from build123d import *

# Parameters (mm, degrees)
BASE_PLATE_184X82X17_DEPTH      = 17
BEARING_SADDLE_DEPTH            = 45
RAISED_PAD_DEPTH                = 82
STEP_PROFILE_DEPTH              = 82
SLOT_CUT_DEPTH                  = 82
BOLT_BOSSES_SKETCH_R            = 9
BOLT_BOSSES_2X_WITH_HOLES_DEPTH = 39
END_BLOCK_DEPTH                 = 26


with BuildPart() as part:
    # Base Plate Sketch → Base Plate 184x82x17 (new body)
    with BuildSketch(Plane(origin=(0, 0, 0), x_dir=(1, 0, 0), z_dir=(0, 1, 0))):
        with BuildLine():
            Line((-86, -41), (92, -41))
            Line((92, -41), (92, 41))
            Line((92, 41), (-86, 41))
            ThreePointArc((-86, 41), (-90.242640687, 39.242640687), (-92, 35))
            Line((-92, 35), (-92, -35))
            ThreePointArc((-92, -35), (-90.242640687, -39.242640687), (-86, -41))
        make_face()
    extrude(amount=BASE_PLATE_184X82X17_DEPTH)

    # Bearing Saddle Sketch → Bearing Saddle (add)
    with BuildSketch(Plane(origin=(0, 17, 0), x_dir=(1, 0, 0), z_dir=(0, 1, 0))):
        with BuildLine():
            Line((92, -41), (56, -41))
            ThreePointArc((56, -41), (51.757359313, -39.242640687), (50, -35))
            Line((50, -35), (50, 35))
            ThreePointArc((50, 35), (51.757359313, 39.242640687), (56, 41))
            Line((56, 41), (92, 41))
            Line((92, 41), (92, -41))
        make_face()
    extrude(amount=BEARING_SADDLE_DEPTH)

    # Raised Pad Sketch → Raised Pad (add)
    with BuildSketch(Plane.XY.offset(41)):
        with BuildLine():
            Line((-58, 17), (-58, 0))
            Line((-58, 0), (-38, 0))
            Line((-38, 0), (-38, 17))
            ThreePointArc((-38, 17), (-48, 27), (-58, 17))
        make_face()
    extrude(amount=-RAISED_PAD_DEPTH)

    # Step Profile Sketch → Step Profile (add)
    with BuildSketch(Plane.XY.offset(41)):
        with BuildLine():
            Line((-64, 17), (-58, 17))
            ThreePointArc((-58, 17), (-48, 27), (-38, 17))
            Line((-38, 17), (-32, 17))
            ThreePointArc((-32, 17), (-48, 33), (-64, 17))
        make_face()
    extrude(amount=-STEP_PROFILE_DEPTH)

    # Slot Cut Sketch → Slot Cut (cut)
    with BuildSketch(Plane.XY.offset(41)):
        with BuildLine():
            Line((-58, 17), (-58, 0))
            Line((-58, 0), (-38, 0))
            Line((-38, 0), (-38, 17))
            ThreePointArc((-38, 17), (-48, 27), (-58, 17))
        make_face()
    extrude(amount=-SLOT_CUT_DEPTH, mode=Mode.SUBTRACT)

    # Bolt Bosses Sketch → Bolt Bosses 2x with Holes (add)
    # profile 1 of 2: a face of its own
    with BuildSketch(Plane(origin=(0, 17, 0), x_dir=(1, 0, 0), z_dir=(0, 1, 0))):
        with BuildLine():
            Line((32, 41), (56, 41))
            Line((56, 41), (56, 5))
            Line((56, 5), (32, 5))
            ThreePointArc((32, 5), (14, 23), (32, 41))
        make_face()
        with Locations(Location((32, 23, 0), (0, 0, 270))):
            Circle(BOLT_BOSSES_SKETCH_R, mode=Mode.SUBTRACT)
    # profile 2 of 2: a face of its own
    with BuildSketch(Plane(origin=(0, 17, 0), x_dir=(1, 0, 0), z_dir=(0, 1, 0))):
        with BuildLine():
            Line((32, -5), (56, -5))
            Line((56, -5), (56, -41))
            Line((56, -41), (32, -41))
            ThreePointArc((32, -41), (14, -23), (32, -5))
        make_face()
        with Locations(Location((32, -23, 0), (0, 0, 270))):
            Circle(BOLT_BOSSES_SKETCH_R, mode=Mode.SUBTRACT)
    extrude(amount=BOLT_BOSSES_2X_WITH_HOLES_DEPTH)

    # End Block Sketch → End Block (add, symmetric)
    with BuildSketch(Plane.XY):
        with BuildLine():
            Line((-83, 17), (-64, 17))
            ThreePointArc((-64, 17), (-48, 33), (-32, 17))
            Line((-32, 17), (-13, 17))
            ThreePointArc((-13, 17), (-48, 52), (-83, 17))
        make_face()
    extrude(amount=END_BLOCK_DEPTH, both=True)


solid = part.part
Could you check a few things on this model? Use its own coordinates, in mm. A direction names the side the tool comes from. Give positions to 0.01 mm unless a question says otherwise; leave off trailing zeros. Order: outer loops, then holes, each group sorted by start corner. A loop starts at its lowest first (then second) coordinate and runs counter-clockwise, first axis right, second up.
Item 1: For faces 4 (the face through (51.804, 58.958, 39.289)), 5 (the face through (-48, 35, -26)), 6 (the face through (-84, 17, -1)), 7 (the face through (41, 36, -5)), which set-ups out of +Z, -Z, +X, -X, +Y, -Y let a thin tool reach every point of the face, with its end or its side?
Item 2: If we mould it in two halves opening along Z, with no side actions, what happens to faces 1 (the face through (-90.196, 8.381, -39.289)), 2 (the face through (71, 62, -1)), 3 (the face through (50, 51, 0))? For each: pulls with the +Z half, pulls with the -Z half, needs draft (parallel to the pull), parting line crosses it, or undercut.
Item 3: If we section it at A-A, the plane y = 39: Write out the boundary of the cut face in (x, z).
Item 4: I need wall thicknesses on line 1 (X direction, y = 35.5, z = -23); line 2 (X direction, y = 11.5, z = -5); line 3 (X direction, y = 18.5, z = 18.5). Which ranges of each line are inside material? Lowest first, please.
Item 5: If we section it at B-B, the plane z = -23: Write out the boundary of the cut face in (x, y).
Item 6: If we section it at C-C, the plane y = 24: Write out the boundary of the cut face in (x, z).
Item 7: I'm going to push flat-ended pins straight in: pin 1 (23.5 mm diameter, centred on x = 32, z = -23, fed in from +Y); pin 2 (5.5 mm diameter, centred on x = 34.5, z = -26, fed in from +Y); pin 3 (2 mm diameter, centred on y = 44, z = -25, fed in from -X). Where does each tip first touch, or does it pass through?
Item 8: If we section it at D-D, the plane x = -41.5: Write out the boundary of the cut face in (y, z), plus the area to 3 significant figures.
Values:
1. face 4: +Z, -X, +Y
1. face 5: -Z, +Y
1. face 6: -X, +Y
1. face 7: +Y
2. face 1: pulls with the -Z half
2. face 2: needs draft
2. face 3: undercut
3. outline: (-75.22, -26) - (-20.78, -26) - (-20.78, 26) - (-75.22, 26) - close; (32, -41) - (92, -41) - (92, 41) - (32, 41) arc R18 ccw to (32, 5) - (50, 5) - (50, -5) - (32, -5) arc R18 ccw to start; hole circle Ø18 at (32, -23); hole circle Ø18 at (32, 23)
4. line 1: x = -77.71 to -18.29, 14 to 23, 41 to 92
4. line 2: x = -92 to -58, -38 to 92
4. line 3: x = -82.97 to -57.89, -38.11 to -13.03, 14.57 to 24.21, 39.79 to 92
5. outline: (-92, 0) - (-58, 0) - (-58, 17) arc R10 cw to (-38, 17) - (-38, 0) - (92, 0) - (92, 62) - (50, 62) - (50, 56) - (41, 56) - (41, 17) - (23, 17) - (23, 56) - (14, 56) - (14, 17) - (-13, 17) arc R35 ccw to (-83, 17) - (-92, 17) - close
6. outline: (-82.29, -26) - (-62.39, -26) - (-62.39, -41) - (-55.14, -41) - (-55.14, 41) - (-62.39, 41) - (-62.39, 26) - (-82.29, 26) - close; (-40.86, -41) - (-33.61, -41) - (-33.61, -26) - (-13.71, -26) - (-13.71, 26) - (-33.61, 26) - (-33.61, 41) - (-40.86, 41) - close; (32, -41) - (92, -41) - (92, 41) - (32, 41) arc R18 ccw to (32, 5) - (50, 5) - (50, -5) - (32, -5) arc R18 ccw to start; hole circle Ø18 at (32, -23); hole circle Ø18 at (32, 23)
7. pin 1: stops at y = 56
7. pin 2: stops at y = 17
7. pin 3: stops at x = -71.43
8. outline: (24.6, -41) - (31.62, -41) - (31.62, -26) - (51.39, -26) - (51.39, 26) - (31.62, 26) - (31.62, 41) - (24.6, 41) - close
8. area: 1,600 mm2
